Could you check a few things on this model? Use its own coordinates, in mm. A direction names the side the tool comes from. Coordinates: 2 decimals unless noted, no trailing zeros. Write each loop counter-clockwise with the first axis right and the second up, starting at its lowest first coordinate (ties: lowest second). Pieces come first, ordered by that corner, then holes. Notation, with made-up numbers: M 48.5,67.25 L 79.5,67.25 A34 ccw 79.5,97.25 Z; hole C 49.25,76.5 d1. An arc over 180 degrees is marked long. Answer as CSV lines item,"result". Start each with the question number.
Item 1: Suppose I cut it at B-B, the plane x = 0. Write out the boundary of the cut face in (y, z).
Item 2: Suppose I cut it at C-C, the plane z = -3. Write out the boundary of the cut face in (x, y), and give its area (3 significant figures).
Item 3: Suppose I cut it at A-A, the plane y = 245. Write out the boundary of the cut face in (x, z).
Item 4: On a 3-axis mill with a long thin cutter (end or side, diameter ignored), from which of +Z, -Z, +X, -X, +Y, -Y can I reach the whole of each face in a straight line? I mean faces 1 (the flat face through (4, 167, 10)), 2 (the flat face through (-160, 59, 0)). Say none if no direction works.
Item 5: I'm going to push flat-ended pins straight in: P1, Ø3, axis at y = 51.5, z = -1, coming from the +X side; P2, Ø2, axis at y = 98, z = 5, coming from the +X side; P3, Ø1, axis at x = -107.5, z = -3, coming from the +Y side. Where does each tip first touch, or does it pass through?
Item 6: If I drill on line 1 along X through (y, z) = (246.5, -0.5) (3 decimals); line 2 along X through (y, z) = (161.5, -1.25); line 3 along Y through (x, z) = (0, -3), over which ranges is the centre line in solid material (lowest first)? Write a range as [from, to].
Item 7: Suppose I cut it at D-D, the plane x = -251.5. Write out the boundary of the cut face in (y, z).
```python
from build123d import *

# Parameters (mm, degrees)
SKETCH1_R           = 45
SKETCH1_R_2         = 9
BOSS_EXTRUDE1_DEPTH = 10
M10_TAPPED_HOLE1_D  = 8.5


with BuildPart() as part:
    # Sketch1 → Boss-Extrude1 (new, symmetric)
    with BuildSketch(Plane.XY):
        with BuildLine():
            Line((0, 0), (-160, 0))
            Line((-160, 0), (-160, 120))
            ThreePointArc((-160, 120), (-176.357134778, 174.807582481), (-220.077421949, 211.685264693))
            Line((-220.077421949, 211.685264693), (-258.686064049, 228.496652355))
            ThreePointArc((-258.686064049, 228.496652355), (-269.478553593, 245.878413735), (-257.04300386, 262.12527688))
            Line((-257.04300386, 262.12527688), (-92.383397673, 315.421281327))
            ThreePointArc((-92.383397673, 315.421281327), (0, 330), (92.383397673, 315.421281327))
            Line((92.383397673, 315.421281327), (257.04300386, 262.12527688))
            ThreePointArc((257.04300386, 262.12527688), (269.475222772, 245.944121974), (258.80651528, 228.549625097))
            Line((258.80651528, 228.549625097), (195.408248443, 200.390971685))
            ThreePointArc((195.408248443, 200.390971685), (164.925652867, 179.34512904), (144.195283074, 148.647117803))
            Line((144.195283074, 148.647117803), (80, 0))
            Line((80, 0), (0, 0))
        make_face()
        with Locations((0, 245)):
            Circle(SKETCH1_R, mode=Mode.SUBTRACT)
        with Locations((-251.5, 245)):
            Circle(SKETCH1_R_2, mode=Mode.SUBTRACT)
        with Locations((251.5, 245)):
            Circle(SKETCH1_R_2, mode=Mode.SUBTRACT)
    extrude(amount=BOSS_EXTRUDE1_DEPTH, both=True)

    # M10 Tapped Hole1 (through all)
    with Locations(Plane.XY.offset(10)):
        with Locations((-30, 165), (30, 165)):
            Hole(M10_TAPPED_HOLE1_D / 2)


solid = part.part
```
Ans:
1,outline,"M 0,-10 L 200,-10 L 200,10 L 0,10 Z; M 290,-10 L 330,-10 L 330,10 L 290,10 Z"
2,outline,"M -258.69,228.5 L -220.08,211.69 A100 cw -160,120 L -160,0 L 80,0 L 144.2,148.65 A100 cw 195.41,200.39 L 258.81,228.55 A18 ccw 257.04,262.13 L 92.38,315.42 A300 ccw -92.38,315.42 L -257.04,262.13 A18 ccw Z; hole C -251.5,245 d18; hole C 0,245 d90; hole C -30,165 d8.5; hole C 30,165 d8.5; hole C 251.5,245 d18"
2,area,"102,000 mm^2"
3,outline,"M -269.5,-10 L -260.5,-10 L -260.5,10 L -269.5,10 Z; M -242.5,-10 L -45,-10 L -45,10 L -242.5,10 Z; M 45,-10 L 242.5,-10 L 242.5,10 L 45,10 Z; M 260.5,-10 L 269.5,-10 L 269.5,10 L 260.5,10 Z"
4,face 1,"+Z, +X, -X, +Y, -Y"
4,face 2,"+Z, -Z, -X, -Y"
5,P1,"stops at x = 102.89"
5,P2,"stops at x = 122.75"
5,P3,"stops at y = 310.69"
6,line 1,"x = [-269.437, -260.374], [-242.626, -44.975], [44.975, 242.626], [260.374, 269.437]"
6,line 2,"x = [-169.02, -32.41], [-27.59, 27.59], [32.41, 150.89]"
6,line 3,"y = [0, 200], [290, 330]"
7,outline,"M 225.37,-10 L 236,-10 L 236,10 L 225.37,10 Z; M 254,-10 L 263.92,-10 L 263.92,10 L 254,10 Z"
